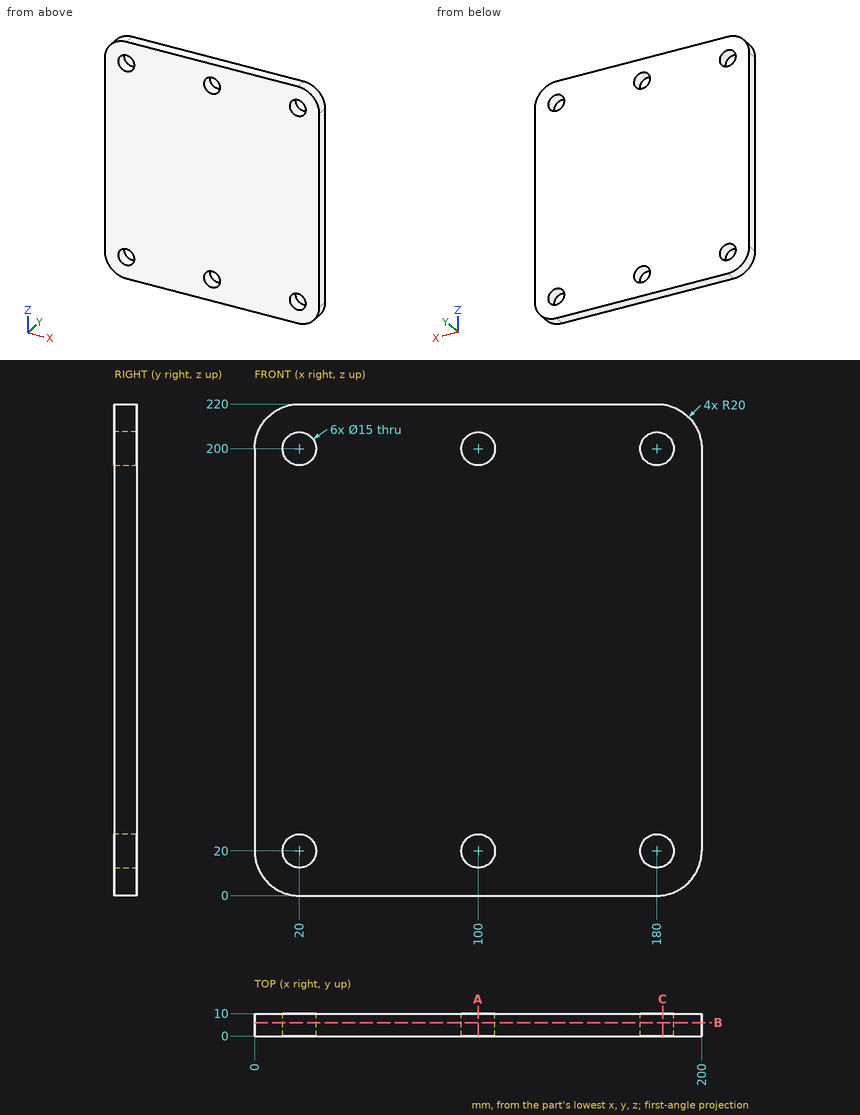
Part print with two shaded views. Sizes in mm from the minimum x, y, z corner. Give positions to 0.01 mm unless a question says otherwise; leave off trailing zeros. Order: outer loops, then holes, each group sorted by start corner. A loop starts at its lowest first (then second) coordinate and runs counter-clockwise, first axis right, second up. Notation, with made-up numbers: M 49.25,-34.75 L 79.25,-34.75 A20 cw 79.25,-5.75 Z; hole C -5.5,12.5 d8. An arc over 180 degrees is marked long. Put each result on its own line as item: value.
Item 1: Wall check: probe 1 along X at (y, z) = (5.5, 20); probe 2 along X at (y, z) = (3.75, 195); probe 3 along Z at (x, y) = (97.5, 4.25). Give the ranges that are in metal, low to high.
Results are:
probe 1: 0 to 12.5, 27.5 to 92.5, 107.5 to 172.5, 187.5 to 200
probe 2: 0 to 14.41, 25.59 to 94.41, 105.59 to 174.41, 185.59 to 200
probe 3: 0 to 12.93, 27.07 to 192.93, 207.07 to 220
Item 2: Cut at B-B on y = 6. Write the cut outline in (x, z), then the cut area to 3 significant figures.
Results are:
outline: M 0,20 A20 ccw 20,0 L 180,0 A20 ccw 200,20 L 200,200 A20 ccw 180,220 L 20,220 A20 ccw 0,200 Z; hole C 20,20 d15; hole C 20,200 d15; hole C 100,20 d15; hole C 100,200 d15; hole C 180,20 d15; hole C 180,200 d15
area: 42,600 mm2
Item 3: Cut at A-A on x = 100. Write the cut outline in (y, z).
Results are:
outline: M 0,0 L 10,0 L 10,12.5 L 0,12.5 Z; M 0,27.5 L 10,27.5 L 10,192.5 L 0,192.5 Z; M 0,207.5 L 10,207.5 L 10,220 L 0,220 Z
Item 4: Cut at C-C on x = 182.5. Write the cut outline in (y, z).
Results are:
outline: M 0,0.16 L 10,0.16 L 10,12.93 L 0,12.93 Z; M 0,27.07 L 10,27.07 L 10,192.93 L 0,192.93 Z; M 0,207.07 L 10,207.07 L 10,219.84 L 0,219.84 Z
